```python
from build123d import *

# Parameters (mm, degrees)
SKETCH1_W               = 100
SKETCH1_H               = 80
BOSS_EXTRUDE1_DEPTH     = 100
CHAMFER1_SIZE           = 10
F_22_DIAMETER_HOLE1_D   = 22
CUT_EXTRUDE1_DEPTH      = 119.74342087
CUT_EXTRUDE1_DEPTH_BACK = 119.74342087


with BuildPart() as part:
    # Sketch1 → Boss-Extrude1 (new body)
    with BuildSketch(Plane.XY):
        Rectangle(SKETCH1_W, SKETCH1_H)
    extrude(amount=BOSS_EXTRUDE1_DEPTH)

    # Chamfer1
    chamfer1_edges = [part.edges().sort_by_distance(p)[0] for p in [
        (-50, 40, 50),
        (50, 40, 50),
    ]]
    chamfer(chamfer1_edges, length=CHAMFER1_SIZE)

    # Ø22 Diameter Hole1 (through all)
    with Locations(Plane.XY.offset(100)):
        with Locations((-27.5, 0), (27.5, 0)):
            Hole(F_22_DIAMETER_HOLE1_D / 2)

    # Sketch4 → Cut-Extrude1 (cut, two sides: drawn at the far end of the back side and taken through both)
    with BuildSketch(Plane.XY.offset(100).offset(-CUT_EXTRUDE1_DEPTH_BACK)):
        Polygon((-35, 40), (-50, 19), (-50, 40), align=None)
        Polygon((50, 40), (35, 40), (50, 19), align=None)
    extrude(amount=CUT_EXTRUDE1_DEPTH + CUT_EXTRUDE1_DEPTH_BACK, mode=Mode.SUBTRACT)


solid = part.part
```
Geometry: final body of the model. Coordinates: model frame, mm. Round coordinates to 2 decimals unless told otherwise and drop trailing zeros. Order: outer loops, then holes, each group sorted by start corner. A loop starts at its lowest first (then second) coordinate and runs counter-clockwise, first axis right, second up. Notation, with made-up numbers: M -8,-14.5 L 24,-14.5 A30 ccw 24,17.5 Z; hole C 38,38 d8. An arc over 180 degrees is marked long. Use one line per item in the form item = value. Start each with the question number.
Q1. Pin query (flat end, axial travel): pin 1 Ø13 at (x, y) = (-27.5, 0) entering from -Z. Return the tip coordinate at first contact, or that it passes through.
Q2. Cut plane D-D (x = 23). Return loops of the section in (y, z).
Q3. Mould query, pull axis X, two halves, no side actions, for faces 1 (the face through (-42.395, 29.647, 49.3)), 2 (the face through (-1, 1, 100)), 3 (the face through (17.339, -4.213, 49.3)). Classes: +X half, -X half, draft (parallel to the pull), parting line (faces both ways), or undercut.
Q4. Material intervals for line 1 (Y direction, x = -27.5, z = 64); line 2 (X direction, y = -0.5, z = 4.5); line 3 (X direction, y = -5.5, z = 90), sorted ascending. Write a range as [from, to].
Q5. Cut plane C-C (z = 14.5). Return loops of the section in (x, y).
Q6. Cut plane A-A (x = -27.5). Return loops of the section in (y, z).
Q7. Cut plane B-B (y = 0). Return loops of the section in (x, z), and give its area (3 significant figures).
Geometry results:
q1.pin_1 = through
q2.outline = M -40,0 L -10.04,0 L -10.04,100 L -40,100 Z; M 10.04,0 L 40,0 L 40,100 L 10.04,100 Z
q3.face_1 = -X half
q3.face_2 = draft
q3.face_3 = undercut
q4.line_1 = [-40, -11], [11, 40]
q4.line_2 = [-50, -38.49], [-16.51, 16.51], [38.49, 50]
q4.line_3 = [-50, -37.03], [-17.97, 17.97], [37.03, 50]
q5.outline = M -50,-40 L 50,-40 L 50,19 L 35,40 L -35,40 L -50,19 Z; hole C -27.5,0 d22; hole C 27.5,0 d22
q6.outline = M -40,0 L -11,0 L -11,100 L -40,100 Z; M 11,0 L 40,0 L 40,100 L 11,100 Z
q7.outline = M -50,0 L -38.5,0 L -38.5,100 L -50,100 Z; M -16.5,0 L 16.5,0 L 16.5,100 L -16.5,100 Z; M 38.5,0 L 50,0 L 50,100 L 38.5,100 Z
q7.area = 5,600 mm^2
